```python
from build123d import *

# Parameters (mm, degrees)
SKETCH_1_W          = 50
SKETCH_1_H          = 50
SKETCH_1_W_2        = 44
SKETCH_1_H_2        = 44
EXTRUDE_1_DEPTH     = 790
SKETCH_2_W          = 50
SKETCH_2_H          = 45
CUT_EXTRUDE_1_DEPTH = 5
SKETCH_3_R          = 5
CUT_EXTRUDE_2_DEPTH = 5
CUT_EXTRUDE_3_DEPTH = 50
CUT_EXTRUDE_4_DEPTH = 50
EXTRUDE_2_DEPTH     = 25
EXTRUDE_3_DEPTH     = 25
CUT_EXTRUDE_5_DEPTH = 25
CUT_EXTRUDE_6_DEPTH = 25
SKETCH_10_R         = 5
CUT_EXTRUDE_7_DEPTH = 94


with BuildPart() as part:
    # 草图1 → 凸台-拉伸1 (new body)
    with BuildSketch(Plane.XY):
        with Locations((25, 25)):
            Rectangle(SKETCH_1_W, SKETCH_1_H)
        with Locations((25, 25)):
            Rectangle(SKETCH_1_W_2, SKETCH_1_H_2, mode=Mode.SUBTRACT)
    extrude(amount=EXTRUDE_1_DEPTH)

    # 草图2 → 切除-拉伸1 (cut)
    with BuildSketch(Plane(origin=(0, 50, 0), x_dir=(1, 0, 0), z_dir=(0, 1, 0))):
        with Locations((25, -22.5)):
            Rectangle(SKETCH_2_W, SKETCH_2_H)
        with Locations((25, -767.5)):
            Rectangle(SKETCH_2_W, SKETCH_2_H)
    extrude(amount=-CUT_EXTRUDE_1_DEPTH, mode=Mode.SUBTRACT)

    # 草图3 → 切除-拉伸2 (cut)
    with BuildSketch(Plane(origin=(0, 50, 0), x_dir=(1, 0, 0), z_dir=(0, 1, 0))):
        with Locations(Location((35, -330, 0), (0, 0, 270))):
            Circle(SKETCH_3_R)
    extrude(amount=-CUT_EXTRUDE_2_DEPTH, mode=Mode.SUBTRACT)

    # 草图4 → 切除-拉伸3 (cut)
    with BuildSketch(Plane.XY.offset(790)):
        Polygon((50, 0), (50, 45), (47, 45), (47, 3), (3, 3), (3, 45), (0, 45), (0, 0), align=None)
    extrude(amount=-CUT_EXTRUDE_3_DEPTH, mode=Mode.SUBTRACT)

    # 草图5 → 切除-拉伸4 (cut)
    with BuildSketch(Plane.XY.offset(745)):
        Polygon((47, 47), (47, 45), (50, 45), (50, 50), (0, 50), (0, 45), (3, 45), (3, 47), align=None)
    extrude(amount=-CUT_EXTRUDE_4_DEPTH, mode=Mode.SUBTRACT)

    # 草图6 → 凸台-拉伸2 (add)
    with BuildSketch(Plane.XY.offset(695)):
        Polygon((3, 47), (47, 47), (47, 45), (50, 45), (50, 50), (0, 50), (0, 45), (3, 45), align=None)
    extrude(amount=EXTRUDE_2_DEPTH)

    # 草图7 → 凸台-拉伸3 (add)
    with BuildSketch(Plane.XY.offset(740)):
        Polygon((0, 0), (50, 0), (50, 45), (47, 45), (47, 3), (3, 3), (3, 45), (0, 45), align=None)
    extrude(amount=EXTRUDE_3_DEPTH)

    # 草图8 → 切除-拉伸5 (cut)
    with BuildSketch(Plane(origin=(0, 0, 0), x_dir=(-1, 0, 0), z_dir=(0, 0, -1))):
        Polygon((0, 0), (0, 45), (-3, 45), (-3, 3), (-47, 3), (-47, 45), (-50, 45), (-50, 0), align=None)
    extrude(amount=-CUT_EXTRUDE_5_DEPTH, mode=Mode.SUBTRACT)

    # 草图9 → 切除-拉伸6 (cut)
    with BuildSketch(Plane(origin=(0, 0, 45), x_dir=(-1, 0, 0), z_dir=(0, 0, -1))):
        Polygon((-47, 45), (-47, 47), (-3, 47), (-3, 45), (0, 45), (0, 50), (-50, 50), (-50, 45), align=None)
    extrude(amount=-CUT_EXTRUDE_6_DEPTH, mode=Mode.SUBTRACT)

    # 草图10 → 切除-拉伸7 (cut)
    with BuildSketch(Plane(origin=(0, 50, 0), x_dir=(1, 0, 0), z_dir=(0, 1, 0))):
        with Locations(Location((35, -330, 0), (0, 0, 270))):
            Circle(SKETCH_10_R)
    extrude(amount=-CUT_EXTRUDE_7_DEPTH, mode=Mode.SUBTRACT)


solid = part.part
```
Work out the finished part from the listing and answer in its coordinate system (mm). A direction names the side the tool comes from. Give positions to 0.01 mm unless a question says otherwise; leave off trailing zeros. Write each loop counter-clockwise with the first axis right and the second up, starting at its lowest first coordinate (ties: lowest second). Pieces come first, ordered by that corner, then holes. Notation, with made-up numbers: (-15, 71.25) - (13, 71.25) arc R28 cw to (13, 93.25) - close; hole circle Ø4 at (28.5, 60.25). An arc over 180 degrees is marked (long way). Use one line per item in the form item = value.
1. Consider L1, parallel to X at y = 14.5, z = 170.5; L2, parallel to X at y = 49, z = 330. Determine where each line is inside the solid, lowest interval first.
Filled in:
L1 = 0 to 3, 47 to 50
L2 = 0 to 30, 40 to 50
2. A cutting plane is placed at C-C (z = 414). Write down the section's boundary in (x, y).
Filled in:
outline = (0, 0) - (50, 0) - (50, 50) - (0, 50) - close; hole (3, 3) - (47, 3) - (47, 47) - (3, 47) - close
3. For faces 4 (the face through (25.1, 2.6, 25)), 5 (the face through (25, 3, 390)), determine the directions among +Z, -Z, +X, -X, +Y, -Y from which every point of the face is accessible in a straight line to the end or side of a thin tool.
Filled in:
face_4 = -Z, +X, -X, +Y, -Y
face_5 = +Z, -Z
4. Determine the mould class of faces 1 (the face through (0, 25, 390)), 2 (the face through (3, 25, 390)), 3 (the face through (25, 0, 390)) for opening direction Y: released by +Y, released by -Y, zero draft, split by the parting line, or undercut.
Filled in:
face_1 = zero draft
face_2 = undercut
face_3 = released by -Y
5. A cutting plane is placed at A-A (x = 23). Write down the section's boundary in (y, z), and give its area (3 significant figures).
Filled in:
outline = (0, 25) - (3, 25) - (3, 765) - (0, 765) - close; (47, 70) - (50, 70) - (50, 720) - (47, 720) - close
area = 4,170 mm^2
6. Each of these flat-tipped pins is pushed along its axis until it touches: pin 1 Ø1.5 at (x, z) = (2, 56) entering from +Y; pin 2 Ø6 at (y, z) = (31.5, 313.5) entering from -X; pin 3 Ø9 at (x, z) = (35, 330) entering from +Y; pin 4 Ø2.5 at (x, y) = (33.5, 47.5) entering from -Z. Where does it stop, or does it pass through?
Filled in:
pin_1 = 45
pin_2 = 0
pin_3 = through
pin_4 = 70
7. A cutting plane is placed at B-B (y = 11.5). Write down the section's boundary in (x, z), and give its area (3 significant figures).
Filled in:
outline = (0, 25) - (3, 25) - (3, 765) - (0, 765) - close; (47, 25) - (50, 25) - (50, 765) - (47, 765) - close
area = 4,440 mm^2
